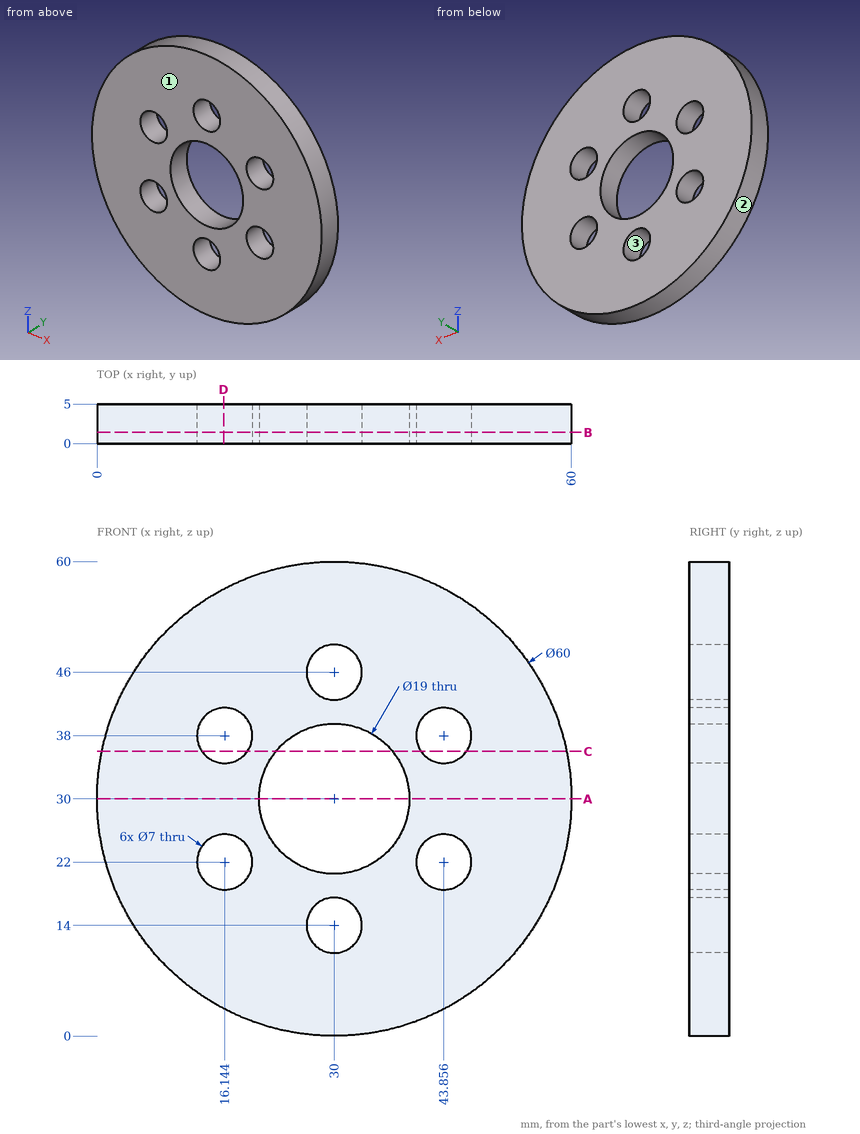
Drawing for the job (mm, zero at the part's lowest x, y, z). Give positions to 0.01 mm unless a question says otherwise; leave off trailing zeros. Order: outer loops, then holes, each group sorted by start corner. A loop starts at its lowest first (then second) coordinate and runs counter-clockwise, first axis right, second up. Notation, with made-up numbers: M -16,26.25 L 16,26.25 A13 cw 16,50.25 Z; hole C 28.5,-28 d2. An arc over 180 degrees is marked long. Use a Markdown table: item, result. Add a question column.
(1) Mould opens along Z. For the marked faces 1, 2 and 3 say: +Z half, -Z half, draft (parallel to the pull), parting line (faces both ways), or undercut.
(2) Saw through at B-B, the plane y = 1.4. Give the cut face in (x, z), and give its area (3 significant figures).
(3) Drop a flat-ended pin along its axis: P1, Ø1, axis at y = 0.5, z = 23.5, coming from the -X side. Give the stop position or say it passes through.
(4) Saw through at C-C, the plane z = 36. Give the cut face in (x, y) (1 decimal).
(5) Saw through at D-D, the plane x = 16. Give the cut face in (y, z), and give its area (3 significant figures).
(6) Saw through at A-A, the plane z = 30. Give the cut face in (x, y), and give its area (3 significant figures).
(7) Probe line 1 along X through (y, z) = (3.2, 38) (1 decimal); line 2 along X through (y, z) = (2.5, 30); line 3 along Z through (x, y) = (29.5, 3.45) (1 decimal). List the from-to ranges inside material, lowest first. Write a range as [from, to].
Answer key:
| question | item | result |
|---|---|---|
| 1 | face 1 | draft |
| 1 | face 2 | parting line |
| 1 | face 3 | undercut |
| 2 | outline | C 30,30 d60; hole C 16.14,22 d7; hole C 16.14,38 d7; hole C 30,30 d19; hole C 30,14 d7; hole C 30,46 d7; hole C 43.86,22 d7; hole C 43.86,38 d7 |
| 2 | area | 2,310 mm^2 |
| 3 | P1 | x = 0.61 |
| 4 | outline | M 0.6,0 L 13.3,0 L 13.3,5 L 0.6,5 Z; M 19,0 L 22.6,0 L 22.6,5 L 19,5 Z; M 37.4,0 L 41,0 L 41,5 L 37.4,5 Z; M 46.7,0 L 59.4,0 L 59.4,5 L 46.7,5 Z |
| 5 | outline | M 0,3.47 L 5,3.47 L 5,18.5 L 0,18.5 Z; M 0,25.5 L 5,25.5 L 5,34.5 L 0,34.5 Z; M 0,41.5 L 5,41.5 L 5,56.53 L 0,56.53 Z |
| 5 | area | 195 mm^2 |
| 6 | outline | M 0,0 L 20.5,0 L 20.5,5 L 0,5 Z; M 39.5,0 L 60,0 L 60,5 L 39.5,5 Z |
| 6 | area | 205 mm^2 |
| 7 | line 1 | [1.1, 12.6], [19.6, 24.9], [35.1, 40.4], [47.4, 58.9] |
| 7 | line 2 | [0, 20.5], [39.5, 60] |
| 7 | line 3 | [0, 10.5], [17.5, 20.5], [39.5, 42.5], [49.5, 60] |
